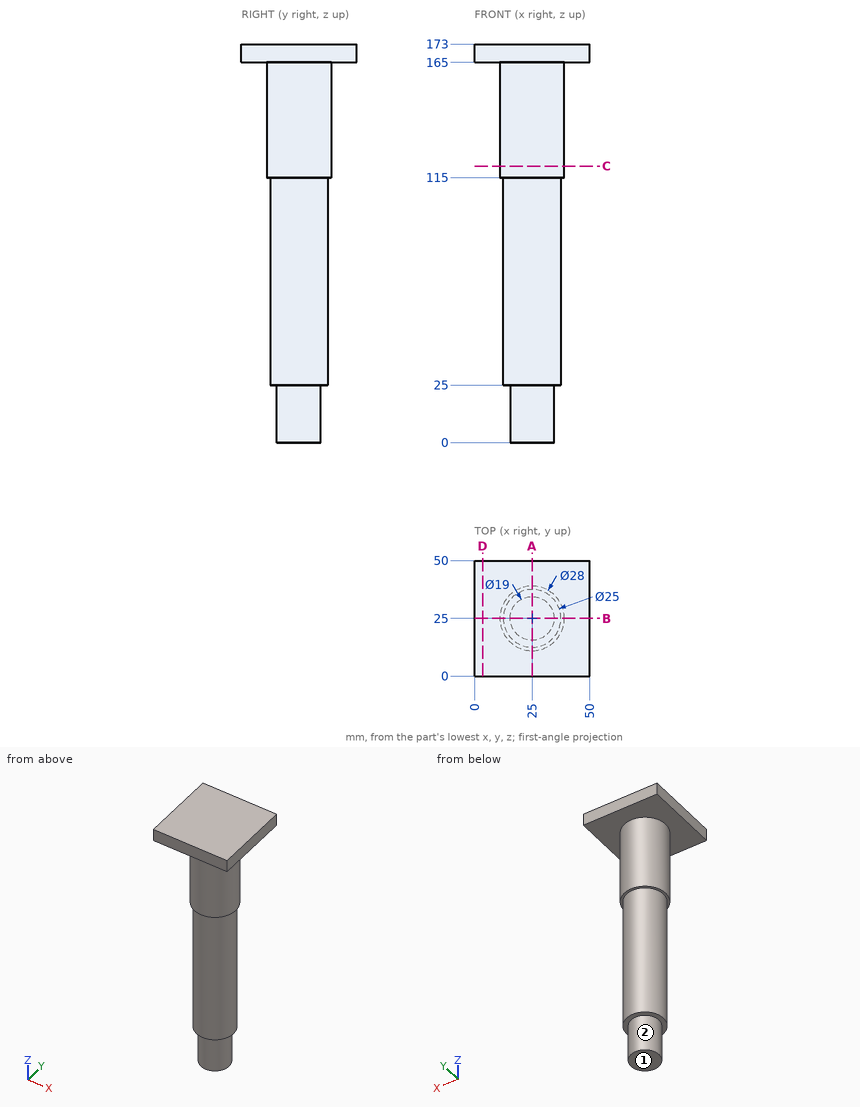
Job drawing, mm, ordinate dimensions from the low corner. One solid piece. A direction names the side the tool comes from. Give positions to 0.01 mm unless a question says otherwise; leave off trailing zeros. Loops run counter-clockwise (first coordinate to the right, second up) from the corner with the lowest first, then second, coordinate; pieces in that order, holes last. Notation, with made-up numbers: M 55.5,16 L 102.5,16 A14 ccw 102.5,42 Z; hole C 27,37 d7. An arc over 180 degrees is marked long. Answer in a Markdown table with one row per item. Add a question column.
Item 1: Drop flat-ended pins along their axis: P1, Ø12, axis at x = 32.5, y = 23.5, coming from the -Z side; P2, Ø12, axis at x = 22.5, z = 81, coming from the -Y side; P3, Ø5, axis at x = 25, z = 30, coming from the +Y side; P4, Ø10, axis at x = 20.5, z = 142.5, coming from the -Y side. Give the stop position or say it passes through.
Item 2: Tool access for the marked faces 1 and 2: list every direction of +Z, -Z, +X, -X, +Y, -Y with a clear straight run to the whole face (end or side of a thin tool).
Item 3: Band-saw the part on D-D on x = 3.5. Give the cut face in (y, z).
Item 4: Probe probe 1 along Z at (x, y) = (36.5, 35); probe 2 along Z at (x, y) = (32, 18.5); probe 3 along X at (y, z) = (25.5, 101.5). List the from-to ranges inside material, lowest first.
Item 5: Band-saw the part on C-C on z = 120. Give the cut face in (x, y).
Item 6: Band-saw the part on A-A on x = 25. Give the cut face in (y, z).
Reply:
| question | item | result |
|---|---|---|
| 1 | P1 | stops at z = 0 |
| 1 | P2 | stops at y = 12.5 |
| 1 | P3 | stops at y = 37.5 |
| 1 | P4 | stops at y = 11 |
| 2 | face 1 | -Z, +X, -X, +Y, -Y |
| 2 | face 2 | -Z |
| 3 | outline | M 0,165 L 50,165 L 50,173 L 0,173 Z |
| 4 | probe 1 | z = 165 to 173 |
| 4 | probe 2 | z = 25 to 173 |
| 4 | probe 3 | x = 12.51 to 37.49 |
| 5 | outline | C 25,25 d28 |
| 6 | outline | M 0,165 L 11,165 L 11,115 L 12.5,115 L 12.5,25 L 15.5,25 L 15.5,0 L 34.5,0 L 34.5,25 L 37.5,25 L 37.5,115 L 39,115 L 39,165 L 50,165 L 50,173 L 0,173 Z |
